from build123d import *

# Parameters (mm, degrees)
BASE_PLATE_SKETCH_W          = 200
BASE_PLATE_SKETCH_H          = 100
BASE_PLATE_200X100X30_DEPTH  = 15
PLATE_END_CHAMFERS_10MM_SIZE = 10
PIN_HOLES_SKETCH_R           = 7.5
PIN_HOLES_SKETCH_R_2         = 15
PIN_HOLES_SKETCH_R_3         = 22.5
PIN_HOLES_15_30_45_DEPTH     = 30
PIN_HOLE_CHAMFERS_5MM_SIZE   = 5


with BuildPart() as part:
    # Base Plate Sketch → Base Plate 200x100x30 (new, symmetric)
    with BuildSketch(Plane(origin=(0, 0, 0), x_dir=(1, 0, 0), z_dir=(0, 1, 0))):
        Rectangle(BASE_PLATE_SKETCH_W, BASE_PLATE_SKETCH_H)
    extrude(amount=BASE_PLATE_200X100X30_DEPTH, both=True)

    # Plate End Chamfers 10mm
    plate_end_chamfers_10mm_edges = [part.edges().sort_by_distance(p)[0] for p in [
        (-100, 15, 0),
        (0, 15, 50),
        (100, 15, 0),
        (0, -15, 50),
        (-100, -15, 0),
        (0, -15, -50),
        (100, -15, 0),
        (0, 15, -50),
    ]]
    chamfer(plate_end_chamfers_10mm_edges, length=PLATE_END_CHAMFERS_10MM_SIZE)

    # Pin Holes Sketch → Pin Holes Ø15 Ø30 Ø45 (cut)
    with BuildSketch(Plane(origin=(0, 15, 0), x_dir=(1, 0, 0), z_dir=(0, 1, 0))):
        with Locations(Location((-75, 0, 0), (0, 0, 270))):
            Circle(PIN_HOLES_SKETCH_R)
        with Locations(Location((-25, 0, 0), (0, 0, 270))):
            Circle(PIN_HOLES_SKETCH_R_2)
        with Locations(Location((50, 0, 0), (0, 0, 270))):
            Circle(PIN_HOLES_SKETCH_R_3)
    extrude(amount=-PIN_HOLES_15_30_45_DEPTH, mode=Mode.SUBTRACT)

    # Pin Hole Chamfers 5mm
    pin_hole_chamfers_5mm_edges = [part.edges().sort_by_distance(p)[0] for p in [
        (-75, 15, -7.5),
        (-25, 15, -15),
        (50, 15, -22.5),
    ]]
    chamfer(pin_hole_chamfers_5mm_edges, length=PIN_HOLE_CHAMFERS_5MM_SIZE)


solid = part.part
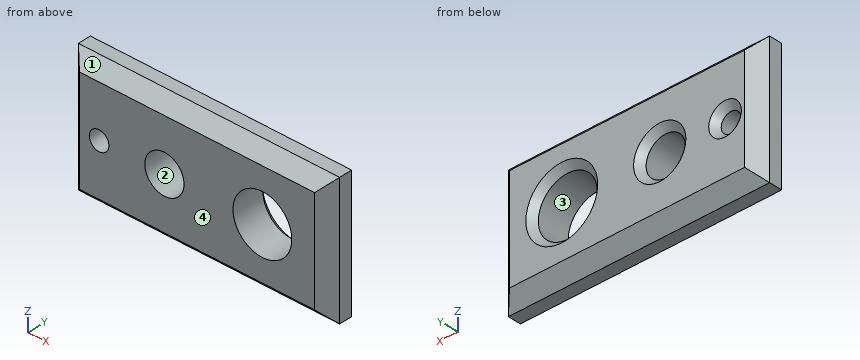
For this review, take the finished solid that the model builds, in its own axes (mm). Face numbers are marked on the shaded views. Round coordinates to 2 decimals unless told otherwise and drop trailing zeros. Write each loop counter-clockwise with the first axis right and the second up, starting at its lowest first coordinate (ties: lowest second). Pieces come first, ordered by that corner, then holes. Notation, with made-up numbers: (87.25, -30.5) - (102.25, -30.5) arc R25 cw to (102.25, -7.5) - close; hole circle Ø1 at (66, 75.5). An arc over 180 degrees is marked (long way). Use a Markdown table: item, result.
Q1. The part is to be moulded in two halves that separate along Z. For the marked faces 1, 2, 3 and 4, say which applies: pulls with the +Z half, pulls with the -Z half, needs draft (parallel to the pull), parting line crosses it, or undercut.
Derived:
| item | result |
|---|---|
| face 1 | pulls with the +Z half |
| face 2 | undercut |
| face 3 | undercut |
| face 4 | needs draft |
Q2. We need section A-A (x = -25). Give the boundary of the cut face in (y, z), plus the area to 4 significant figures.
Derived:
| item | result |
|---|---|
| outline | (-15, -40) - (-5, -50) - (5, -50) - (15, -40) - (15, -20) - (10, -15) - (-15, -15) - close; (-15, 15) - (10, 15) - (15, 20) - (15, 40) - (5, 50) - (-5, 50) - (-15, 40) - close |
| area | 1,875 mm2 |
Q3. We need section B-B (y = -11). Give the boundary of the cut face in (x, z), plus the area to 3 significant figures.
Derived:
| item | result |
|---|---|
| outline | (-94, -44) - (94, -44) - (94, 44) - (-94, 44) - close; hole circle Ø15 at (-75, 0); hole circle Ø30 at (-25, 0); hole circle Ø45 at (50, 0) |
| area | 14,100 mm2 |
Q4. We need section C-C (x = -75). Give the boundary of the cut face in (y, z).
Derived:
| item | result |
|---|---|
| outline | (-15, -40) - (-5, -50) - (5, -50) - (15, -40) - (15, -12.5) - (10, -7.5) - (-15, -7.5) - close; (-15, 7.5) - (10, 7.5) - (15, 12.5) - (15, 40) - (5, 50) - (-5, 50) - (-15, 40) - close |
Q5. We need section D-D (x = 17). Give the boundary of the cut face in (y, z), plus the area to 3 significant figures.
Derived:
| item | result |
|---|---|
| outline | (-15, -40) - (-5, -50) - (5, -50) - (15, -40) - (15, 40) - (5, 50) - (-5, 50) - (-15, 40) - close |
| area | 2,800 mm2 |
Q6. Wall thickness on line 1 along X through (y, z) = (4.25, 0); line 2 along X through (y, z) = (-5.5, -13); line 3 along X through (y, z) = (1.5, 6): over which ranges is each line inside the solid? List them lowest first.
Derived:
| item | result |
|---|---|
| line 1 | x = -100 to -82.5, -67.5 to -40, -10 to 27.5, 72.5 to 100 |
| line 2 | x = -99.5 to -32.48, -17.52 to 31.64, 68.36 to 99.5 |
| line 3 | x = -100 to -79.5, -70.5 to -38.75, -11.25 to 28.31, 71.69 to 100 |
Q7. Clearance check with flat-ended pins moving along their axes: pin 1 (5 mm diameter, centred on y = 11, z = -7.5, fed in from +X); pin 2 (1.5 mm diameter, centred on x = 31.5, y = -8, fed in from -Z). State where each tip first meets the part, or that it passes through.
Derived:
| item | result |
|---|---|
| pin 1 | stops at x = 96.5 |
| pin 2 | stops at z = -47.75 |
